from build123d import *

# Parameters (mm, degrees)
SKETCH1_W           = 100
SKETCH1_H           = 130
BOSS_EXTRUDE1_DEPTH = 5
F_12_HOLE1_D        = 12


with BuildPart() as part:
    # Sketch1 → Boss-Extrude1 (new, symmetric)
    with BuildSketch(Plane.XY):
        Rectangle(SKETCH1_W, SKETCH1_H)
    extrude(amount=BOSS_EXTRUDE1_DEPTH, both=True)

    # Ø12 Hole1 (through all)
    with Locations(Plane.XY.offset(5)):
        with Locations((-40, 40), (40, 40), (40, -40), (-40, -40)):
            Hole(F_12_HOLE1_D / 2)


solid = part.part
For this review, take the finished solid that the model builds, in its own axes (mm). Coordinates: 2 decimals unless noted, no trailing zeros. Order: outer loops, then holes, each group sorted by start corner. A loop starts at its lowest first (then second) coordinate and runs counter-clockwise, first axis right, second up. Notation, with made-up numbers: (15, 13) - (22, 13) arc R17 ccw to (22, 30) - close; hole circle Ø8 at (61.5, -21.5). An arc over 180 degrees is marked (long way). Answer as CSV lines item,"result". Start each with the question number.
1) Add section A-A (x = -40). State the section outline as (y, z) points, then the cut area to 3 significant figures.
2) Add section B-B (y = 40). State the section outline as (x, z) points.
3) To check wall thickness, follow line 1 along Y through (x, z) = (40, 1.25); line 2 along Y through (x, z) = (-41.5, 4). State the ranges of each line that lie inside material, in increasing order. Write a range as [from, to].
4) Draft analysis for pull direction Y (two halves, no side actions). For faces 1 (the flat face through (-1, -65, 0)), 2 (the flat face through (-1, 1, 5)), 3 (the cylindrical face through (-35.24, 36.35, -0.07)), state which applies: +Y half, -Y half, draft (parallel to the pull), parting line (faces both ways), or undercut.
5) Add section C-C (z = -3.25). State the section outline as (x, y) points.
6) Insertion check: P1, Ø7, axis at x = -40, y = -40, coming from the -Z side. The pin has a flat end and moves straight along its axis. Give the tip position at first contact, or say it passes through.
Result:
1,outline,"(-65, -5) - (-46, -5) - (-46, 5) - (-65, 5) - close; (-34, -5) - (34, -5) - (34, 5) - (-34, 5) - close; (46, -5) - (65, -5) - (65, 5) - (46, 5) - close"
1,area,"1,060 mm^2"
2,outline,"(-50, -5) - (-46, -5) - (-46, 5) - (-50, 5) - close; (-34, -5) - (34, -5) - (34, 5) - (-34, 5) - close; (46, -5) - (50, -5) - (50, 5) - (46, 5) - close"
3,line 1,"[-65, -46], [-34, 34], [46, 65]"
3,line 2,"[-65, -45.81], [-34.19, 34.19], [45.81, 65]"
4,face 1,"-Y half"
4,face 2,"draft"
4,face 3,"undercut"
5,outline,"(-50, -65) - (50, -65) - (50, 65) - (-50, 65) - close; hole circle Ø12 at (-40, -40); hole circle Ø12 at (-40, 40); hole circle Ø12 at (40, -40); hole circle Ø12 at (40, 40)"
6,P1,"through"
